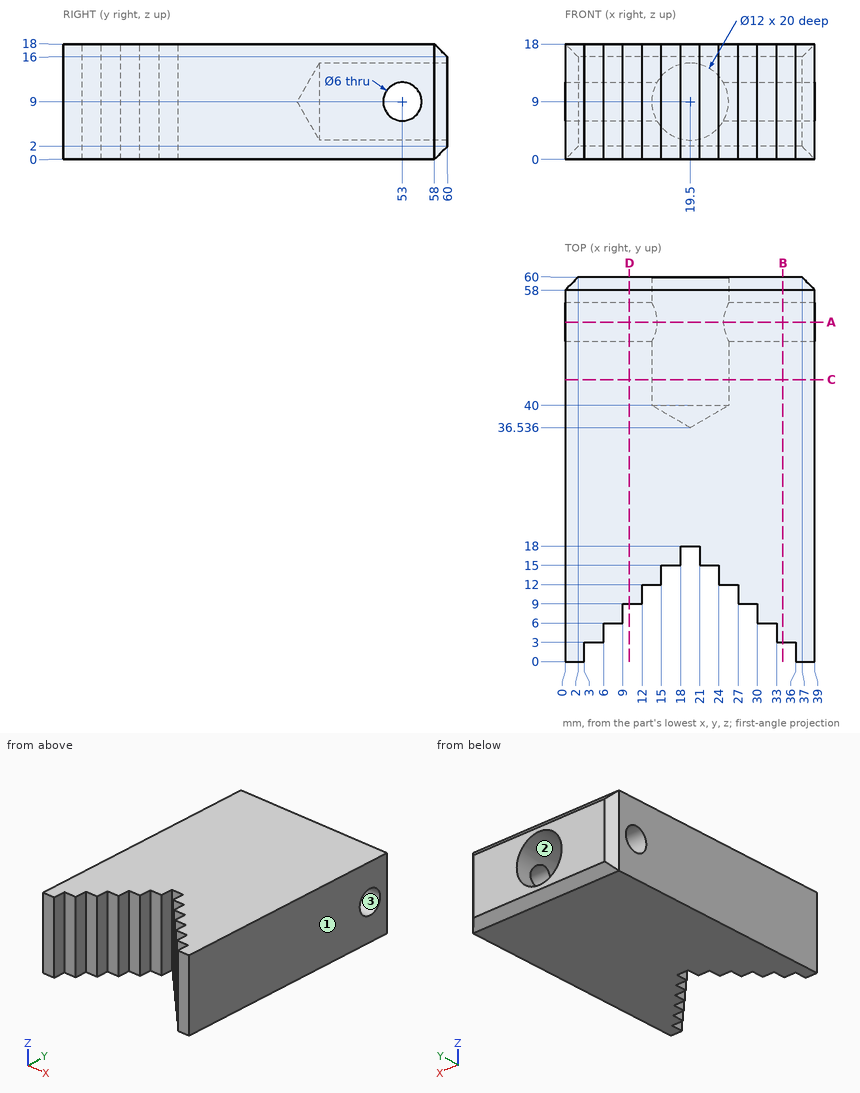
Here's the drawing with two shaded views (mm, measured from the low corner). I have some questions. Coordinates: 2 decimals unless noted, no trailing zeros. Order: outer loops, then holes, each group sorted by start corner. A loop starts at its lowest first (then second) coordinate and runs counter-clockwise, first axis right, second up. Notation, with made-up numbers: (-24.75, 86) - (-13.75, 86) arc R11 ccw to (-13.75, 90) - close; hole circle Ø1 at (26.5, 46). An arc over 180 degrees is marked (long way). Answer in a Markdown table with one row per item.
1. Suppose I cut it at B-B (x = 34). Please give me the cut outline in (y, z), and give its area (3 significant figures).
Reply:
| item | result |
|---|---|
| outline | (3, 0) - (58, 0) - (60, 2) - (60, 16) - (58, 18) - (3, 18) - close; hole circle Ø6 at (53, 9) |
| area | 994 mm^2 |
2. Suppose I cut it at A-A (y = 53). Please give me the cut outline in (x, z).
Reply:
| item | result |
|---|---|
| outline | (0, 0) - (39, 0) - (39, 6) - (24.7, 6) arc R6 cw to (14.3, 6) - (0, 6) - close; (0, 12) - (14.3, 12) arc R6 cw to (24.7, 12) - (39, 12) - (39, 18) - (0, 18) - close |
3. Suppose I cut it at C-C (y = 44). Please give me the cut outline in (x, z), and give its area (3 significant figures).
Reply:
| item | result |
|---|---|
| outline | (0, 0) - (39, 0) - (39, 18) - (0, 18) - close; hole circle Ø12 at (19.5, 9) |
| area | 589 mm^2 |
4. If I drill on line 1 along X through (y, z) = (11, 3.25); line 2 along Y through (x, z) = (26.5, 9.25); line 3 along Z through (x, y) = (5, 53), over which ranges is the centre line in solid material (lowest first)?
Reply:
| item | result |
|---|---|
| line 1 | x = 0 to 12, 27 to 39 |
| line 2 | y = 12 to 50.01, 55.99 to 60 |
| line 3 | z = 0 to 6, 12 to 18 |
5. Suppose I cut it at D-D (x = 10). Please give me the cut outline in (y, z), and give its area (3 significant figures).
Reply:
| item | result |
|---|---|
| outline | (9, 0) - (58, 0) - (60, 2) - (60, 16) - (58, 18) - (9, 18) - close; hole circle Ø6 at (53, 9) |
| area | 886 mm^2 |
6. If we mould it in two halves opening along X, with no side actions, what happens to the marked faces 1, 2 and 3? For each: pulls with the +X half, pulls with the -X half, needs draft (parallel to the pull), parting line crosses it, or undercut.
Reply:
| item | result |
|---|---|
| face 1 | pulls with the +X half |
| face 2 | undercut |
| face 3 | needs draft |
7. For pin 1 (2.5 mm diameter, centred on x = 25.5, z = 8.5, fed in from -Y); pin 2 (3.5 mm diameter, centred on x = 31, z = 7.5, fed in from -Y); pin 3 (5 mm diameter, centred on y = 53, z = 9, fed in from -X); pin 4 (3.5 mm diameter, centred on x = 34, z = 13, fed in from -Y), each with a flat end and sliding along its axis, tell me the tip position at first contact or that it passes through.
Reply:
| item | result |
|---|---|
| pin 1 | stops at y = 12 |
| pin 2 | stops at y = 6 |
| pin 3 | passes through |
| pin 4 | stops at y = 3 |
